The figure shows three views and two pictorial views of one solid part (mm, origin at its lowest corner). Answer the questions. Give positions to 0.01 mm unless a question says otherwise; leave off trailing zeros. Write item = value, one per line. Start each with the question number.
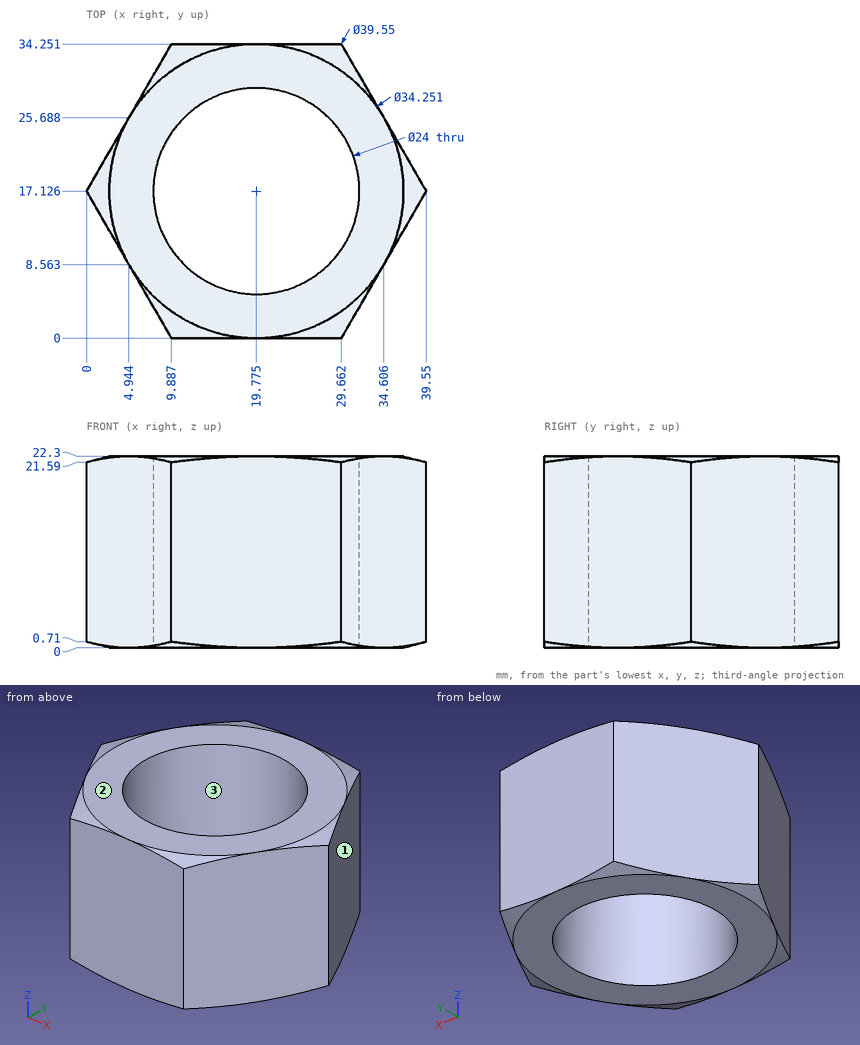
(1) Determine the mould class of the marked faces 1, 2 and 3 for opening direction X: pulls with the +X half, pulls with the -X half, needs draft (parallel to the pull), parting line crosses it, or undercut.
(2) Each of these flat-tipped pins is pushed along its axis until it touches: pin 1 (1 mm diameter, centred on x = 31.5, z = 2.5, fed in from +Y) (1 decimal); pin 2 (6 mm diameter, centred on x = 34.5, z = 5.5, fed in from +Y); pin 3 (14.5 mm diameter, centred on x = 19.77, y = 17.13, fed in from -Z); pin 4 (6 mm diameter, centred on y = 6.5, z = 12, fed in from +X). Where does it stop, or does it pass through?
(3) Find the intervals of material crossed by line 1 along X through (y, z) = (10, 7) (1 decimal); line 2 along X through (y, z) = (18, 13) (1 decimal); line 3 along Y through (x, z) = (25, 12.75), in increasing order.
Results list:
q1.face_1 = pulls with the +X half
q1.face_2 = needs draft
q1.face_3 = undercut
q2.pin_1 = 31.9
q2.pin_2 = 31.07
q2.pin_3 = through
q2.pin_4 = 35.15
q3.line_1 = 4.1 to 10.1, 29.4 to 35.4
q3.line_2 = 0.5 to 7.8, 31.7 to 39
q3.line_3 = 0 to 6.32, 27.93 to 34.25
